```python
from build123d import *

# Parameters (mm, degrees)
SKETCH_1_W                   = 110
SKETCH_1_H                   = 175
EXTRUDE_1_DEPTH              = 6
CHAMFER_1_SIZE               = 50
CHAMFER_1_SIZE2              = 120
CHAMFER_2_SIZE               = 65
CHAMFER_2_SIZE2              = 120
HOLE_WIZARD_M5_1_D           = 5
HOLE_WIZARD_M5_1_2_D         = 4.2
F_5_0MM_1_D                  = 5
HOLE_WIZARD_M5_3_D           = 5.5
HOLE_WIZARD_M5_3_CBORE_D     = 9.8
HOLE_WIZARD_M5_3_CBORE_DEPTH = 5.4
HOLE_WIZARD_M5_4_D           = 5.5
HOLE_WIZARD_M5_4_CBORE_D     = 10
HOLE_WIZARD_M5_4_CBORE_DEPTH = 5.4
HOLE_WIZARD_M4_1_D           = 4.5
HOLE_WIZARD_M4_1_CBORE_D     = 8
HOLE_WIZARD_M4_1_CBORE_DEPTH = 4.4
HOLE_WIZARD_M5_6_D           = 5.5
HOLE_WIZARD_M5_6_CBORE_D     = 9.8
HOLE_WIZARD_M5_6_CBORE_DEPTH = 5.4
SKETCH_16_W                  = 20
SKETCH_16_H                  = 12
CUT_EXTRUDE_1_DEPTH          = 105.04446165
FILLET_1_R                   = 2.5


with BuildPart() as part:
    # 草图1 → 凸台-拉伸1 (new, symmetric)
    with BuildSketch(Plane.XY):
        Rectangle(SKETCH_1_W, SKETCH_1_H)
    extrude(amount=EXTRUDE_1_DEPTH, both=True)

    # 倒角1
    chamfer_1_edges = [part.edges().sort_by_distance(p)[0] for p in [
        (-55, 87.5, 0),
    ]]
    chamfer_1_side = [part.faces().sort_by_distance(p)[0] for p in [
        (0, 87.5, 0),
    ]]
    chamfer(chamfer_1_edges, length=CHAMFER_1_SIZE, length2=CHAMFER_1_SIZE2, reference=chamfer_1_side[0])

    # 倒角2
    chamfer_2_edges = [part.edges().sort_by_distance(p)[0] for p in [
        (55, -87.5, 0),
    ]]
    chamfer_2_side = [part.faces().sort_by_distance(p)[0] for p in [
        (0, -87.5, 0),
    ]]
    chamfer(chamfer_2_edges, length=CHAMFER_2_SIZE, length2=CHAMFER_2_SIZE2, reference=chamfer_2_side[0])

    # Hole Wizard M5 _1 (through all)
    with Locations(Plane.XY.offset(6)):
        with Locations((47.5, 82.5), (2.5, 82.5)):
            Hole(HOLE_WIZARD_M5_1_D / 2)

    # Hole Wizard M5 _1 2 (through all)
    with Locations(Plane.XY.offset(6)):
        with Locations((0, 30), (25.980762114, 15), (25.980762114, -15), (0, -30), (-25.980762114, -15), (-25.980762114, 15)):
            Hole(HOLE_WIZARD_M5_1_2_D / 2)

    # Ø5.0mm 暗销孔1 (through all)
    with Locations(Plane.XY.offset(6)):
        with Locations((30, 0), (-30, 0)):
            Hole(F_5_0MM_1_D / 2)

    # M5 六角凹头螺钉的柱形沉头孔3 (through all)
    with Locations(Plane.XY.offset(6)):
        with Locations((38, 82.5), (12, 82.5)):
            CounterBoreHole(HOLE_WIZARD_M5_3_D / 2, HOLE_WIZARD_M5_3_CBORE_D / 2, HOLE_WIZARD_M5_3_CBORE_DEPTH)

    # M5 六角凹头螺钉的柱形沉头孔4 (through all)
    with Locations(Plane.XY.offset(6)):
        with Locations((15, 67.5), (15, 47.5)):
            CounterBoreHole(HOLE_WIZARD_M5_4_D / 2, HOLE_WIZARD_M5_4_CBORE_D / 2, HOLE_WIZARD_M5_4_CBORE_DEPTH)

    # M4 六角凹头螺钉的柱形沉头孔1 (through all)
    with Locations(Plane.XY.offset(6)):
        with Locations((-45, -56), (-23, -56)):
            CounterBoreHole(HOLE_WIZARD_M4_1_D / 2, HOLE_WIZARD_M4_1_CBORE_D / 2, HOLE_WIZARD_M4_1_CBORE_DEPTH)

    # M5 六角凹头螺钉的柱形沉头孔6 (through all)
    with Locations(Plane.XY.offset(6)):
        with Locations((-50, -64.75), (-18, -82.75)):
            CounterBoreHole(HOLE_WIZARD_M5_6_D / 2, HOLE_WIZARD_M5_6_CBORE_D / 2, HOLE_WIZARD_M5_6_CBORE_DEPTH)

    # 草图16 → 切除-拉伸1 (cut, through all)
    with BuildSketch(Plane.XY.offset(6)):
        with Locations((-34, -87.5)):
            Rectangle(SKETCH_16_W, SKETCH_16_H)
    extrude(amount=-CUT_EXTRUDE_1_DEPTH, mode=Mode.SUBTRACT)

    # 圆角1
    fillet_1_edges = [part.edges().sort_by_distance(p)[0] for p in [
        (-24, -81.5, 0),
        (-44, -81.5, 0),
    ]]
    fillet(fillet_1_edges, radius=FILLET_1_R)


solid = part.part
```
Geometry check sheet. Reference: the model listing, model coordinates, mm. A direction names the side the tool comes from. Coordinates: 2 decimals unless noted, no trailing zeros. Write each loop counter-clockwise with the first axis right and the second up, starting at its lowest first coordinate (ties: lowest second). Pieces come first, ordered by that corner, then holes. Notation, with made-up numbers: M 25.25,-9.5 L 53.25,-9.5 A20 cw 53.25,11.5 Z; hole C 85,83.25 d4. An arc over 180 degrees is marked long. Answer as a JSON object with one key per item and string values.
1. Draft check along Y on faces 3 (the cylindrical face through (-47.973, -62.891, -2.746)), 4 (the flat face through (25, 87.5, 0)). Enter one of: released by +Y, released by -Y, zero draft, split by the parting line, or undercut.
Answers below:
{"face 3": "undercut", "face 4": "released by +Y"}
2. Section check B-B, the plane y = 0. Enter the section's corners in (x, z), plus the area to 3 significant figures.
Answers below:
{"outline": "M -41.46,-6 L -32.5,-6 L -32.5,6 L -41.46,6 Z; M -27.5,-6 L 27.5,-6 L 27.5,6 L -27.5,6 Z; M 32.5,-6 L 37.4,-6 L 37.4,6 L 32.5,6 Z", "area": "826 mm²"}
3. Section check D-D, the plane y = 67.5. Enter the section's corners in (x, z).
Answers below:
{"outline": "M -13.33,-6 L 12.25,-6 L 12.25,0.6 L 10,0.6 L 10,6 L -13.33,6 Z; M 17.75,-6 L 55,-6 L 55,6 L 20,6 L 20,0.6 L 17.75,0.6 Z"}
4. Section check A-A, the plane z = -1.75. Give the number of separate pieces and of enclosed holes in the cut face, plus the area to 3 significant figures.
Answers below:
{"separate pieces": "1", "enclosed holes": "18", "area": "11,900 mm²"}
5. Scan lines: L1, parallel to Y at x = 14.5, z = 2.25; L2, parallel to Y at x = 1.5, z = 0.75; L3, parallel to Y at x = 30.5, z = -2. Record each from-to range of solid material in increasing order.
Answers below:
{"L1": "y = -42.27 to 42.53, 52.47 to 62.53, 72.47 to 78.29, 86.71 to 87.5", "L2": "y = -66.27 to -31.47, -28.53 to 28.53, 31.47 to 80.21, 84.79 to 87.5", "L3": "y = -12.73 to -2.45, 2.45 to 87.5"}
6. Tool access check on faces 1 (the cylindrical face through (-45.867, -59.905, 3.831)), 2 (the cylindrical face through (2.83, 84.98, -0.08)). Record the directions out of +Z, -Z, +X, -X, +Y, -Y that give a thin tool (end or side, any length) a straight path to the whole face; none if there is none.
Answers below:
{"face 1": "+Z", "face 2": "+Z, -Z"}
7. Go/stop test with flat-tipped pins: pin 1 Ø7 at (x, y) = (-18, -82.75) entering from -Z; pin 2 Ø4 at (y, z) = (-14, 3) entering from -X (3 decimals); pin 3 Ø6.5 at (x, y) = (38, 82.5) entering from +Z; pin 4 Ø1.5 at (y, z) = (-42.5, 2.5) entering from +X. Record where each tip stops, or that it passes through.
Answers below:
{"pin 1": "stops at z = -6", "pin 2": "stops at x = -48.125", "pin 3": "stops at z = 0.6", "pin 4": "stops at x = 14.78"}
8. Section check C-C, the plane x = 38. Enter the section's corners in (y, z), plus the area to 3 significant figures.
Answers below:
{"outline": "M 1.12,-6 L 79.75,-6 L 79.75,0.6 L 77.6,0.6 L 77.6,6 L 1.12,6 Z; M 85.25,-6 L 87.5,-6 L 87.5,6 L 87.4,6 L 87.4,0.6 L 85.25,0.6 Z", "area": "947 mm²"}
